The listing builds one solid part. Answer for the finished solid, in the listing's coordinates (mm). Round coordinates to 2 decimals unless told otherwise and drop trailing zeros. Write each loop counter-clockwise with the first axis right and the second up, starting at its lowest first coordinate (ties: lowest second). Pieces come first, ordered by that corner, then holes. Notation, with made-up numbers: (35, -38.5) - (47, -38.5) arc R15 cw to (47, -12.5) - close; hole circle Ø9 at (43, -15.75). An arc over 180 degrees is marked (long way). Answer in a Markdown table with one row per item.
from build123d import *

# Parameters (mm, degrees)
SKETCH_1_W            = 98
SKETCH_1_H            = 100
EXTRUDE_1_DEPTH       = 10
HOLE_WIZARD_9_0_9_1_D = 9


with BuildPart() as part:
    # 草图1 → 凸台-拉伸1 (new body)
    with BuildSketch(Plane(origin=(0, 0, 0), x_dir=(0, 0, -1), z_dir=(1, 0, 0))):
        Rectangle(SKETCH_1_W, SKETCH_1_H)
    extrude(amount=EXTRUDE_1_DEPTH)

    # Ø9.0 (9) 直径孔1 (through all)
    with Locations(Plane(origin=(10, 0, 0), x_dir=(0, 0, -1), z_dir=(1, 0, 0))):
        with Locations((-39, 30), (39, 30), (-39, -30), (39, -30)):
            Hole(HOLE_WIZARD_9_0_9_1_D / 2)


solid = part.part
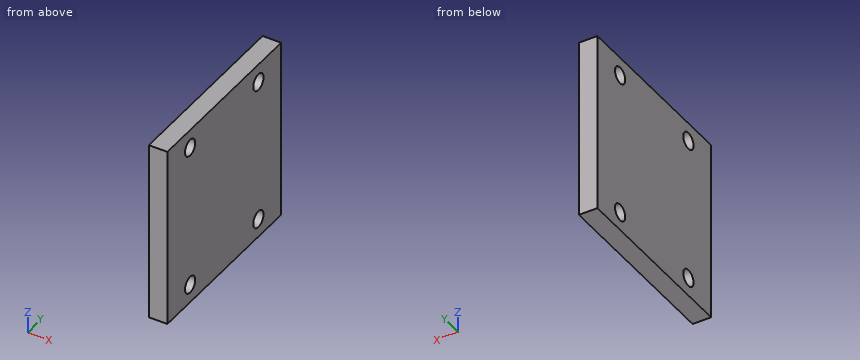
(1) Section B-B (z = -39) is taken. Give the vertices of the cut face in (x, y).
Checked values:
| item | result |
|---|---|
| outline | (0, -50) - (10, -50) - (10, -34.5) - (0, -34.5) - close; (0, -25.5) - (10, -25.5) - (10, 25.5) - (0, 25.5) - close; (0, 34.5) - (10, 34.5) - (10, 50) - (0, 50) - close |
(2) Section A-A (y = -30) is taken. Give the vertices of the cut face in (x, z), and give its area (3 significant figures).
Checked values:
| item | result |
|---|---|
| outline | (0, -49) - (10, -49) - (10, -43.5) - (0, -43.5) - close; (0, -34.5) - (10, -34.5) - (10, 34.5) - (0, 34.5) - close; (0, 43.5) - (10, 43.5) - (10, 49) - (0, 49) - close |
| area | 800 mm2 |
(3) Find the intervals of material crossed by line 1 (Y direction, x = 7.5, z = 39); line 2 (Y direction, x = 5.5, z = 42); line 3 (Z direction, x = 8.25, y = -27), in increasing order.
Checked values:
| item | result |
|---|---|
| line 1 | y = -50 to -34.5, -25.5 to 25.5, 34.5 to 50 |
| line 2 | y = -50 to -33.35, -26.65 to 26.65, 33.35 to 50 |
| line 3 | z = -49 to -42.35, -35.65 to 35.65, 42.35 to 49 |
(4) A flat-ended cylindrical pin translates along its axis: pin 1 (5.5 mm diameter, centred on y = -30, z = -39, fed in from +X). Find the tip coordinate at first contact, or state that the pin passes through.
Checked values:
| item | result |
|---|---|
| pin 1 | passes through |
(5) Section C-C (x = 4.5) is taken. Give the vertices of the cut face in (y, z).
Checked values:
| item | result |
|---|---|
| outline | (-50, -49) - (50, -49) - (50, 49) - (-50, 49) - close; hole circle Ø9 at (-30, -39); hole circle Ø9 at (-30, 39); hole circle Ø9 at (30, -39); hole circle Ø9 at (30, 39) |
